Work out the finished part from the listing and answer in its coordinate system (mm). Coordinates: 2 decimals unless noted, no trailing zeros. Order: outer loops, then holes, each group sorted by start corner. A loop starts at its lowest first (then second) coordinate and runs counter-clockwise, first axis right, second up.
1. A flat-ended cylindrical pin translates along its axis: pin 1 Ø23.5 at (x, z) = (-70, -150) entering from +Y. Find the tip coordinate at first contact, or state that the pin passes through.
2. The part is cut by section A-A, the plane z = -150. Give the vertices of the cut face in (x, y), then the cut area to 3 significant figures.
3. The part is cut by section B-B, the plane x = -70. Give the vertices of the cut face in (y, z).
4. Find the intervals of material crossed by probe 1 along X at (y, z) = (12.5, -151); probe 2 along Z at (x, y) = (-70, 14.5); probe 3 along Z at (x, y) = (-64, 10.75), in increasing order.
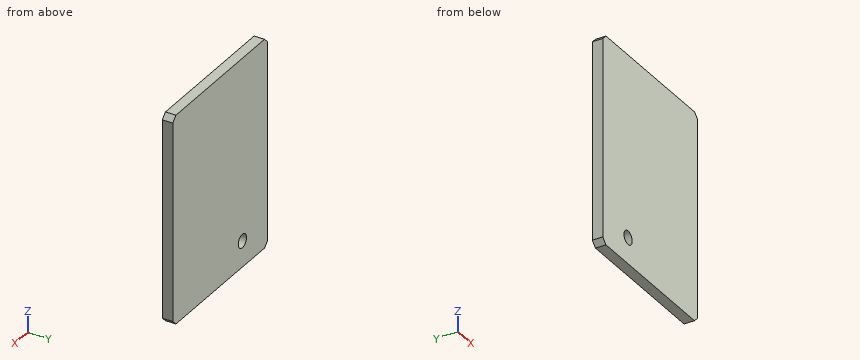
```python
from build123d import *

# Parameters (mm, degrees)
SKETCH_1_W          = 300
SKETCH_1_H          = 400
EXTRUDE_1_DEPTH     = 20
CHAMFER_1_SIZE      = 10
HOLE_WIZARD_M24_1_D = 26


with BuildPart() as part:
    # 草图1 → 凸台-拉伸1 (new body)
    with BuildSketch(Plane(origin=(0, 0, 0), x_dir=(1, 0, 0), z_dir=(0, 1, 0))):
        Rectangle(SKETCH_1_W, SKETCH_1_H)
    extrude(amount=EXTRUDE_1_DEPTH)

    # 倒角1
    chamfer_1_edges = [part.edges().sort_by_distance(p)[0] for p in [
        (150, 10, 200),
        (-150, 10, 200),
        (-150, 10, -200),
        (150, 10, -200),
    ]]
    chamfer(chamfer_1_edges, length=CHAMFER_1_SIZE)

    # M24 间隙孔1 (through all)
    with Locations(Plane(origin=(0, 0, 0), x_dir=(-1, 0, 0), z_dir=(0, -1, 0))):
        with Locations((70, 150)):
            Hole(HOLE_WIZARD_M24_1_D / 2)


solid = part.part
```
Geometry says:
1. pin 1: passes through
2. outline: (-150, 0) - (-83, 0) - (-83, 20) - (-150, 20) - close; (-57, 0) - (150, 0) - (150, 20) - (-57, 20) - close
2. area: 5,480 mm2
3. outline: (0, -200) - (20, -200) - (20, -163) - (0, -163) - close; (0, -137) - (20, -137) - (20, 200) - (0, 200) - close
4. probe 1: x = -150 to -82.96, -57.04 to 150
4. probe 2: z = -200 to -163, -137 to 200
4. probe 3: z = -200 to -161.53, -138.47 to 200
